Geometry: final body of the model. Coordinates: model frame, mm. A direction names the side the tool comes from. Round coordinates to 2 decimals unless told otherwise and drop trailing zeros. Loops run counter-clockwise (first coordinate to the right, second up) from the corner with the lowest first, then second, coordinate; pieces in that order, holes last. Notation, with made-up numbers: (78, -7.5) - (123, -7.5) arc R8 ccw to (123, 3.5) - close; hole circle Ø4 at (-14, 87.25). An arc over 180 degrees is marked (long way). Answer as CSV lines item,"result".
from build123d import *

# Parameters (mm, degrees)
SKETCH_1_W                = 300
SKETCH_1_H                = 100
EXTRUDE_1_DEPTH           = 10
HOLE_WIZARD_1_D           = 6.6
HOLE_WIZARD_1_CBORE_D     = 11
HOLE_WIZARD_1_CBORE_DEPTH = 6.8
HOLE_WIZARD_M8_1_D        = 9
CHAMFER_1_SIZE            = 30


with BuildPart() as part:
    # 草图1 → 凸台-拉伸1 (new body)
    with BuildSketch(Plane.XY):
        Rectangle(SKETCH_1_W, SKETCH_1_H)
    extrude(amount=EXTRUDE_1_DEPTH)

    # 打孔尺寸(%根据)内六角圆柱头螺钉的类型1 (through all)
    with Locations(Plane(origin=(0, 0, 0), x_dir=(-1, 0, 0), z_dir=(0, 0, -1))):
        with Locations((32.599999971, -37.5), (-32.400000029, -37.5), (-32.400000029, 37.5), (32.599999971, 37.5)):
            CounterBoreHole(HOLE_WIZARD_1_D / 2, HOLE_WIZARD_1_CBORE_D / 2, HOLE_WIZARD_1_CBORE_DEPTH)

    # M8 间隙孔1 (through all)
    with Locations(Plane(origin=(0, 0, 0), x_dir=(-1, 0, 0), z_dir=(0, 0, -1))):
        with Locations((-130, 0), (130, 0)):
            Hole(HOLE_WIZARD_M8_1_D / 2)

    # 倒角1
    chamfer_1_edges = [part.edges().sort_by_distance(p)[0] for p in [
        (-150, 50, 5),
        (150, 50, 5),
        (150, -50, 5),
        (-150, -50, 5),
    ]]
    chamfer(chamfer_1_edges, length=CHAMFER_1_SIZE)


solid = part.part
(1) Access query for faces 5 (the face through (135, 35, 5)), 6 (the face through (27.154, -35.848, 3.352)). Directions: +Z, -Z, +X, -X, +Y, -Y. A direction counts if a zero-diameter tool reaches every point of the face in a straight line with its end or side. Return the directions, or none.
Findings below:
face 5,"+Z, -Z, +X, +Y"
face 6,"-Z"
(2) Section B-B (z = 2.75). Output: boundary loops of the cut face in (x, y), and give its area (3 significant figures).
Findings below:
outline,"(-150, -20) - (-120, -50) - (120, -50) - (150, -20) - (150, 20) - (120, 50) - (-120, 50) - (-150, 20) - close; hole circle Ø9 at (-130, 0); hole circle Ø11 at (-32.6, -37.5); hole circle Ø11 at (-32.6, 37.5); hole circle Ø11 at (32.4, -37.5); hole circle Ø11 at (32.4, 37.5); hole circle Ø9 at (130, 0)"
area,"27,700 mm2"
(3) Section D-D (x = 130). Output: boundary loops of the cut face in (y, z), and give its area (3 significant figures).
Findings below:
outline,"(-40, 0) - (-4.5, 0) - (-4.5, 10) - (-40, 10) - close; (4.5, 0) - (40, 0) - (40, 10) - (4.5, 10) - close"
area,"710 mm2"
(4) Section A-A (y = 0). Output: boundary loops of the cut face in (x, z), and give its area (3 significant figures).
Findings below:
outline,"(-150, 0) - (-134.5, 0) - (-134.5, 10) - (-150, 10) - close; (-125.5, 0) - (125.5, 0) - (125.5, 10) - (-125.5, 10) - close; (134.5, 0) - (150, 0) - (150, 10) - (134.5, 10) - close"
area,"2,820 mm2"
(5) Material intervals for line 1 along Y through (x, z) = (-32.6, 3.75); line 2 along Y through (x, z) = (-32.6, 8.25); line 3 along X through (y, z) = (1, 9), sorted ascending.
Findings below:
line 1,"-50 to -43, -32 to 32, 43 to 50"
line 2,"-50 to -40.8, -34.2 to 34.2, 40.8 to 50"
line 3,"-150 to -134.39, -125.61 to 125.61, 134.39 to 150"
(6) Draft query along Y for faces 1 (the face through (-35, -40, 6.8)), 2 (the face through (-150, 0, 5)), 3 (the face through (-2, -50, 5)), 4 (the face through (35.55, -36.51, 8.42)). Return one class per face: pulls with the +Y half, pulls with the -Y half, needs draft (parallel to the pull), parting line crosses it, or undercut.
Findings below:
face 1,"undercut"
face 2,"needs draft"
face 3,"pulls with the -Y half"
face 4,"undercut"
(7) Pin query (flat end, axial travel): P1, Ø3.5, axis at x = 32, y = 38.5, coming from the -Z side; P2, Ø9, axis at x = -32.6, y = 37.5, coming from the -Z side; P3, Ø4, axis at y = 25.5, z = 7.5, coming from the +X side. Return the tip coordinate at first contact, or that it passes through.
Findings below:
P1,"through"
P2,"z = 6.8"
P3,"x = 146.5"
(8) Section C-C (x = 32.4). Output: boundary loops of the cut face in (y, z).
Findings below:
outline,"(-50, 0) - (-43, 0) - (-43, 6.8) - (-40.8, 6.8) - (-40.8, 10) - (-50, 10) - close; (-34.2, 6.8) - (-32, 6.8) - (-32, 0) - (32, 0) - (32, 6.8) - (34.2, 6.8) - (34.2, 10) - (-34.2, 10) - close; (40.8, 6.8) - (43, 6.8) - (43, 0) - (50, 0) - (50, 10) - (40.8, 10) - close"
